```python
from build123d import *

# Parameters (mm, degrees)
EXTRUDE_1_DEPTH     = 17.5
CUT_EXTRUDE_1_DEPTH = 14
CUT_EXTRUDE_2_DEPTH = 47.706530593
CUT_EXTRUDE_3_DEPTH = 58.22979993


with BuildPart() as part:
    # 草图1 → 凸台-拉伸1 (new, symmetric)
    with BuildSketch(Plane.XY):
        Polygon((-22.5, 0), (-22.5, 3.5), (14, 40), (17.5, 40), (17.5, 0), align=None)
    extrude(amount=EXTRUDE_1_DEPTH, both=True)

    # 草图2 → 切除-拉伸1 (cut, symmetric)
    with BuildSketch(Plane.XY):
        Polygon((14.5, 3), (14.5, 49.29015486), (-34.195136802, 3), align=None)
    extrude(amount=CUT_EXTRUDE_1_DEPTH, both=True, mode=Mode.SUBTRACT)

    # 草图4 → 切除-拉伸2 (cut, through all)
    with BuildSketch(Plane(origin=(0, 3, 0), x_dir=(1, 0, 0), z_dir=(0, 1, 0))):
        with BuildLine():
            Line((-11.5, 4.75), (4.5, 4.75))
            ThreePointArc((4.5, 4.75), (9.25, 0), (4.5, -4.75))
            Line((4.5, -4.75), (-11.5, -4.75))
            ThreePointArc((-11.5, -4.75), (-16.25, 0), (-11.5, 4.75))
        make_face()
    extrude(amount=-CUT_EXTRUDE_2_DEPTH, mode=Mode.SUBTRACT)

    # 草图5 → 切除-拉伸3 (cut, through all)
    with BuildSketch(Plane.ZY.offset(-14.5)):
        with BuildLine():
            Line((-4.75, 13), (-4.75, 29))
            ThreePointArc((-4.75, 29), (0, 33.75), (4.75, 29))
            Line((4.75, 29), (4.75, 13))
            ThreePointArc((4.75, 13), (0, 8.25), (-4.75, 13))
        make_face()
    extrude(amount=-CUT_EXTRUDE_3_DEPTH, mode=Mode.SUBTRACT)


solid = part.part
```
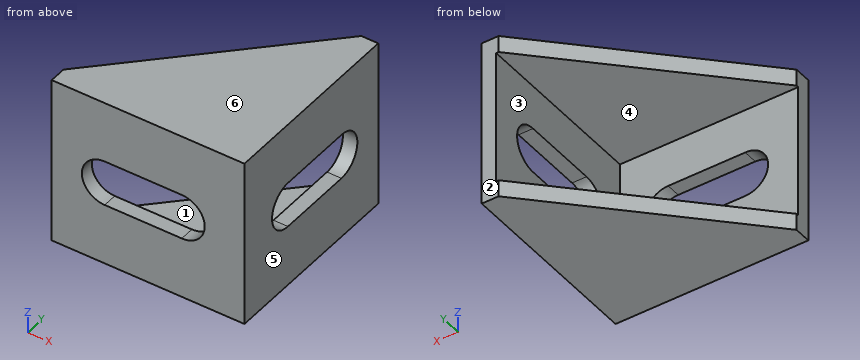
The listing builds one solid part. Answer for the finished solid, in the listing's coordinates (mm). Face numbers are marked on the shaded views. A direction names the side the tool comes from. Coordinates: 2 decimals unless noted, no trailing zeros. Write each loop counter-clockwise with the first axis right and the second up, starting at its lowest first coordinate (ties: lowest second). Pieces come first, ordered by that corner, then holes. Notation, with made-up numbers: (49.5, 31) - (62.5, 31) arc R32 ccw to (62.5, 62) - close; hole circle Ø2 at (-32.5, 51). An arc over 180 degrees is marked (long way). Return JSON: item names as keys, results as strings. Group by question number.
Q1. Find the intervals of material crossed by line 1 along Z through (x, y) = (8, 10); line 2 along X through (y, z) = (12.5, -8.5); line 3 along Y through (x, z) = (-18, -10), in increasing order. Write a range as [from, to].
Q2. The part is cut by section C-C on y = 32. Write down the section's boundary in (x, z), and give its area (3 significant figures).
Q3. The part is cut by section B-B on x = -7.5. Write down the section's boundary in (y, z).
Q4. The part is cut by section D-D on x = -17.5. Write down the section's boundary in (y, z), and give its area (4 significant figures).
Q5. Which of the six approach directions +Z, -Z, +X, -X, +Y, -Y give full straight-line access (tool end or side, diameter ignored) to the marked faces 1 and 2?
Q6. Flat-ended cylindrical pins translate along their axes: pin 1 Ø2 at (y, z) = (20, 10.5) entering from -X; pin 2 Ø8 at (x, z) = (-13, 13) entering from +Y; pin 3 Ø8.5 at (x, z) = (-5, 7) entering from +Y. Find the tip coordinate at first contact, or state that the pin passes through.
Q7. For a pull along Z with two mould halves and no side action, classify the marked faces 3, 4, 5 and 6 as +Z half, -Z half, draft (parallel to the pull), parting line (faces both ways), or undercut.
Q8. The part is cut by section A-A on z = 0. Write down the section's boundary in (x, y), and give its area (3 significant figures).
Evaluation:
{
 "1": {"line 1": "z = [-17.5, -14], [14, 17.5]", "line 2": "x = [14.5, 17.5]", "line 3": "y = [0, 3]"},
 "2": {"outline": "(6, -17.5) - (17.5, -17.5) - (17.5, -3.68) - (14.5, -3.68) - (14.5, -14) - (6, -14) - close; (6, 14) - (14.5, 14) - (14.5, 3.68) - (17.5, 3.68) - (17.5, 17.5) - (6, 17.5) - close", "area": "142 mm2"},
 "3": {"outline": "(0, -17.5) - (18.5, -17.5) - (18.5, -14) - (3, -14) - (3, -4.75) - (0, -4.75) - close; (0, 4.75) - (3, 4.75) - (3, 14) - (18.5, 14) - (18.5, 17.5) - (0, 17.5) - close"},
 "4": {"outline": "(0, -17.5) - (8.5, -17.5) - (8.5, -14) - (3, -14) - (3, 14) - (8.5, 14) - (8.5, 17.5) - (0, 17.5) - close", "area": "143.5 mm2"},
 "5": {"face 1": "-X, +Y", "face 2": "+Z, -Z, +X, -X, +Y"},
 "6": {"pin 1": "stops at x = 14.5", "pin 2": "stops at y = 16.87", "pin 3": "stops at y = 3"},
 "7": {"face 3": "undercut", "face 4": "undercut", "face 5": "draft", "face 6": "+Z half"},
 "8": {"outline": "(-22.5, 0) - (-16.25, 0) - (-16.25, 3) - (-22.5, 3) - close; (9.25, 0) - (17.5, 0) - (17.5, 8.25) - (14.5, 8.25) - (14.5, 3) - (9.25, 3) - close; (14.5, 33.75) - (17.5, 33.75) - (17.5, 40) - (14.5, 40) - close", "area": "78.0 mm2"}
}
